Check sheet for the modelled part. Datum: model origin and axes. Units: mm. A direction names the side the tool comes from. Give positions to 0.01 mm unless a question says otherwise; leave off trailing zeros. Answer in a Markdown table with one row per item. Add a question column.
(1) Thickness scan on L1, parallel to X at y = 0, z = 12; L2, parallel to Z at x = -95, y = 2.25; L3, parallel to X at y = -3.75, z = 1. Record the ranges inside material, lowest first. Write a range as [from, to].
(2) Release check for a two-part mould opening along Z. For faces 6 (the face through (-2, 0, 25)), 7 (the face through (-117.385, 0.751, 16.381)), 8 (the face through (-136.759, -0.424, -0.094)) record: released by +Z, released by -Z, zero draft, split by the parting line, or undercut.
(3) Set-up check for faces 1 (the face through (146.38, -2.44, -0.54)), 2 (the face through (-146.38, -2.44, 0.54)), 3 (the face through (-2, 7.5, 0)), 4 (the face through (155, 3, 0)), 5 (the face through (12.5, 0.1, 16.4)): record each of +Z, -Z, +X, -X, +Y, -Y from which the full face is reachable in a straight line by a thin tool's end or side.
(4) Go/stop test with flat-tipped pins: pin 1 (6 mm diameter, centred on y = 0, z = 0, fed in from -X); pin 2 (2.5 mm diameter, centred on x = -95, z = 0, fed in from -Y); pin 3 (4 mm diameter, centred on x = 135, y = 0, fed in from +Z); pin 4 (4 mm diameter, centred on y = 0, z = 0, fed in from -X). Record where each tip stops, or that it passes through.
```python
from build123d import *

# Parameters (mm, degrees)
SKETCH_1_W             = 310
SKETCH_1_H             = 50
EXTRUDE_1_DEPTH        = 7.5
HOLE_WIZARD_M6_1_D     = 5
HOLE_WIZARD_M6_1_DEPTH = 17
HOLE_WIZARD_M6_1_TIP   = 1.502151548
HOLE_WIZARD_M6_2_D     = 5
HOLE_WIZARD_M6_2_DEPTH = 17
HOLE_WIZARD_M6_2_TIP   = 1.502151548
HOLE_WIZARD_M6_3_D     = 5
HOLE_WIZARD_M6_3_DEPTH = 17
HOLE_WIZARD_M6_3_TIP   = 1.502151548
HOLE_WIZARD_M4_1_D     = 3.3


with BuildPart() as part:
    # 草图1 → 凸台-拉伸1 (new, symmetric)
    with BuildSketch(Plane(origin=(0, 0, 0), x_dir=(1, 0, 0), z_dir=(0, 1, 0))):
        Rectangle(SKETCH_1_W, SKETCH_1_H)
    extrude(amount=EXTRUDE_1_DEPTH, both=True)

    # M6 螺纹孔1
    with Locations(Plane.XY.offset(25)):
        with Locations((-115, 0), (10, 0), (135, 0)):
            Hole(HOLE_WIZARD_M6_1_D / 2, depth=HOLE_WIZARD_M6_1_DEPTH)
            with Locations((0, 0, -(HOLE_WIZARD_M6_1_DEPTH + HOLE_WIZARD_M6_1_TIP / 2))):  # 118° drill point
                Cone(0, HOLE_WIZARD_M6_1_D / 2, HOLE_WIZARD_M6_1_TIP, mode=Mode.SUBTRACT)

    # M6 螺纹孔2
    with Locations(Plane(origin=(155, 0, 0), x_dir=(0, 0, -1), z_dir=(1, 0, 0))):
        with Locations((0, 0)):
            Hole(HOLE_WIZARD_M6_2_D / 2, depth=HOLE_WIZARD_M6_2_DEPTH)
            with Locations((0, 0, -(HOLE_WIZARD_M6_2_DEPTH + HOLE_WIZARD_M6_2_TIP / 2))):  # 118° drill point
                Cone(0, HOLE_WIZARD_M6_2_D / 2, HOLE_WIZARD_M6_2_TIP, mode=Mode.SUBTRACT)

    # M6 螺纹孔3
    with Locations(Plane.ZY.offset(155)):
        with Locations((0, 0)):
            Hole(HOLE_WIZARD_M6_3_D / 2, depth=HOLE_WIZARD_M6_3_DEPTH)
            with Locations((0, 0, -(HOLE_WIZARD_M6_3_DEPTH + HOLE_WIZARD_M6_3_TIP / 2))):  # 118° drill point
                Cone(0, HOLE_WIZARD_M6_3_D / 2, HOLE_WIZARD_M6_3_TIP, mode=Mode.SUBTRACT)

    # M4 螺纹孔1 (through all)
    with Locations(Plane(origin=(0, 7.5, 0), x_dir=(1, 0, 0), z_dir=(0, 1, 0))):
        with Locations((-95, 0), (0, 0), (95, 0)):
            Hole(HOLE_WIZARD_M4_1_D / 2)


solid = part.part
```
Answer below:
| question | item | result |
|---|---|---|
| 1 | L1 | x = [-155, -117.5], [-112.5, 7.5], [12.5, 132.5], [137.5, 155] |
| 1 | L2 | z = [-25, -1.65], [1.65, 25] |
| 1 | L3 | x = [-155, -96.31], [-93.69, -1.31], [1.31, 93.69], [96.31, 155] |
| 2 | face 6 | released by +Z |
| 2 | face 7 | zero draft |
| 2 | face 8 | undercut |
| 3 | face 1 | +X |
| 3 | face 2 | -X |
| 3 | face 3 | +Z, -Z, +X, -X, +Y |
| 3 | face 4 | +Z, -Z, +X, +Y, -Y |
| 3 | face 5 | +Z |
| 4 | pin 1 | stops at x = -155 |
| 4 | pin 2 | passes through |
| 4 | pin 3 | stops at z = 7.7 |
| 4 | pin 4 | stops at x = -137.7 |
